from build123d import *

# Parameters (mm, degrees)
CHAMFER1_SIZE           = 1
CUT_EXTRUDE1_DEPTH      = 95.902265516
CUT_EXTRUDE1_DEPTH_BACK = 95.902265516
SKETCH2_W               = 41.2
SKETCH2_H               = 27.770788335
SKETCH2_H_2             = 30.82392473
SKETCH3_R               = 12.5
CUT_EXTRUDE2_DEPTH      = 5
SKETCH4_R               = 5
CUT_EXTRUDE3_DEPTH      = 19
SKETCH5_R               = 4
CUT_EXTRUDE4_DEPTH      = 10
SKETCH6_R               = 4
CUT_EXTRUDE5_DEPTH      = 13


with BuildPart() as part:
    # Sketch1 → Revolve1 (revolve)
    with BuildSketch(Plane.XY, mode=Mode.PRIVATE) as revolve1_sk:
        with BuildLine():
            Line((0, 26.75), (0, 40))
            Line((0, 40), (-20, 40))
            Line((-20, 40), (-20, 33))
            Line((-20, 33), (-61.2, 33))
            Line((-61.2, 33), (-61.2, 40))
            Line((-61.2, 40), (-76.2, 40))
            Line((-76.2, 40), (-76.2, 26))
            Line((-76.2, 26), (-75.2, 25))
            Line((-75.2, 25), (-65.7, 25))
            Line((-65.7, 25), (-65.7, 20.741987874))
            ThreePointArc((-65.7, 20.741987874), (-58.03253481, 17.787808996), (-52.2, 12))
            Line((-52.2, 12), (-45.1, 12))
            Line((-45.1, 12), (-44.1, 13))
            Line((-44.1, 13), (-44.1, 14.65))
            Line((-44.1, 14.65), (-36, 14.65))
            Line((-36, 14.65), (-5.065925826, 22.938760193))
            Line((-5.065925826, 22.938760193), (-4.1, 24.197579239))
            Line((-4.1, 24.197579239), (-4.1, 25.75))
            Line((-4.1, 25.75), (-1, 25.75))
            Line((-1, 25.75), (0, 26.75))
        make_face()
    revolve(revolve1_sk.sketch.rotate(Axis((23.528076115, 0, 0), (-1, 0, 0)), 90), axis=Axis((23.528076115, 0, 0), (-1, 0, 0)))

    # Chamfer1
    chamfer1_edges = [part.edges().sort_by_distance(p)[0] for p in [
        (0, 0, 40),
        (-20, 0, 40),
        (-61.2, 0, 40),
        (-76.2, 0, 40),
    ]]
    chamfer(chamfer1_edges, length=CHAMFER1_SIZE)

    # Sketch2 → Cut-Extrude1 (cut, two sides: drawn at the far end of the back side and taken through both)
    with BuildSketch(Plane.XY.offset(-CUT_EXTRUDE1_DEPTH_BACK)):
        with Locations((-40.6, 42.385394168)):
            Rectangle(SKETCH2_W, SKETCH2_H)
        with Locations((-40.6, -43.911962365)):
            Rectangle(SKETCH2_W, SKETCH2_H_2)
    extrude(amount=CUT_EXTRUDE1_DEPTH + CUT_EXTRUDE1_DEPTH_BACK, mode=Mode.SUBTRACT)

    # Sketch3 → Cut-Extrude2 (cut)
    with BuildSketch(Plane(origin=(0, 28.5, 0), x_dir=(1, 0, 0), z_dir=(0, 1, 0))):
        with Locations(Location((-40.6, 0, 0), (0, 0, 270))):
            Circle(SKETCH3_R)
    cut_extrude2 = extrude(amount=-CUT_EXTRUDE2_DEPTH, mode=Mode.SUBTRACT)

    # Sketch4 → Cut-Extrude3 (cut)
    with BuildSketch(Plane(origin=(0, 23.5, 0), x_dir=(1, 0, 0), z_dir=(0, 1, 0))):
        with Locations(Location((-40.6, 0, 0), (0, 0, 270))):
            Circle(SKETCH4_R)
    cut_extrude3 = extrude(amount=-CUT_EXTRUDE3_DEPTH, mode=Mode.SUBTRACT)

    # Mirror1: Cut-Extrude2, Cut-Extrude3 across plane
    add(cut_extrude2.mirror(Plane.ZX), mode=Mode.SUBTRACT)
    add(cut_extrude3.mirror(Plane.ZX), mode=Mode.SUBTRACT)

    # Sketch5 → Cut-Extrude4 (cut)
    with BuildSketch(Plane.ZY.offset(76.2)):
        with Locations((-34.097701423, 0)):
            Circle(SKETCH5_R)
    extrude(amount=-CUT_EXTRUDE4_DEPTH, mode=Mode.SUBTRACT)

    # Sketch6 → Cut-Extrude5 (cut)
    with BuildSketch(Plane(origin=(0, 0, 0), x_dir=(0, 0, -1), z_dir=(1, 0, 0))):
        with Locations((34.1, 0)):
            Circle(SKETCH6_R)
    extrude(amount=-CUT_EXTRUDE5_DEPTH, mode=Mode.SUBTRACT)


solid = part.part
Work out the finished part from the listing and answer in its coordinate system (mm). A direction names the side the tool comes from. Round coordinates to 2 decimals unless told otherwise and drop trailing zeros. Order: outer loops, then holes, each group sorted by start corner. A loop starts at its lowest first (then second) coordinate and runs counter-clockwise, first axis right, second up. Notation, with made-up numbers: M -30,2 L -11,2 A17 cw -11,16 Z; hole C 80.25,-34 d5. An arc over 180 degrees is marked long. Put each result on its own line as item: value. Start each with the question number.
Q1. Section B-B, the plane z = 0 is taken. Give the number of separate pieces and of enclosed holes in the cut face, and give its area (3 significant figures).
Q2. Section A-A, the plane x = -29.5 is taken. Write down the section's boundary in (y, z).
Q3. Section C-C, the plane x = -16 is taken. Write down the section's boundary in (y, z).
Q4. For a pull along Y with two mould halves and no side action, classify faces 1 (the flat face through (0, -9.2, 25.5)), 2 (the cylindrical face through (-41, 0, 33)), 3 (the flat face through (-55, 28.5, 0)), 4 (the conical face through (-44.9, -0.2, 12.2)) as pulls with the +Y half, pulls with the -Y half, needs draft (parallel to the pull), parting line crosses it, or undercut.
Q5. Flat-ended cylindrical pins translate along their axes: pin 1 (12 mm diameter, centred on x = -44.5, y = 25, fed in from -Z); pin 2 (12 mm diameter, centred on y = -18.5, z = -5, fed in from -X); pin 3 (5 mm diameter, centred on x = -53.5, z = -32, fed in from -Y). Find the tip coordinate at first contact, or state that the pin passes through.
Q6. A tool of negligible diameter and unlimited length cuts with its end or side. For faces 5 (the flat face through (-66.2, 0, -34)), 6 (the flat face through (-55, -28.5, 0)), 7 (the flat face through (-13, 0, -34)), from which of +Z, -Z, +X, -X, +Y, -Y can it reach the whole face along a straight path? Write none if from no direction.
Q7. Straight lines are drawn through the part: L1, parallel to X at y = 19, z = -29; L2, parallel to Y at x = -47.25, z = 0; L3, parallel to Y at x = -2, z = 0. For each, find the intervals that lie inside material, in ascending order. Write a range as [from, to].
Findings below:
1. separate pieces: 4
1. enclosed holes: 0
1. area: 1,850 mm^2
2. outline: M -28.5,-16.64 A33 ccw 28.5,-16.64 L 28.5,-5.75 L 23.5,-5.75 L 23.5,5.75 L 28.5,5.75 L 28.5,16.64 A33 ccw -28.5,16.64 L -28.5,5.75 L -23.5,5.75 L -23.5,-5.75 L -28.5,-5.75 Z; hole C 0,0 d32.78
3. outline: C 0,0 d80; hole C 0,0 d40.02
4. face 1: needs draft
4. face 2: parting line crosses it
4. face 3: pulls with the +Y half
4. face 4: undercut
5. pin 1: stops at z = -26.98
5. pin 2: stops at x = -75.36
5. pin 3: stops at y = -14.79
6. face 5: -X
6. face 6: +Z, -Z, -Y
6. face 7: +X
7. L1: x = [-76.2, -61.2], [-20, 0]
7. L2: y = [-23.5, -12], [12, 23.5]
7. L3: y = [-40, -25.75], [25.75, 40]
